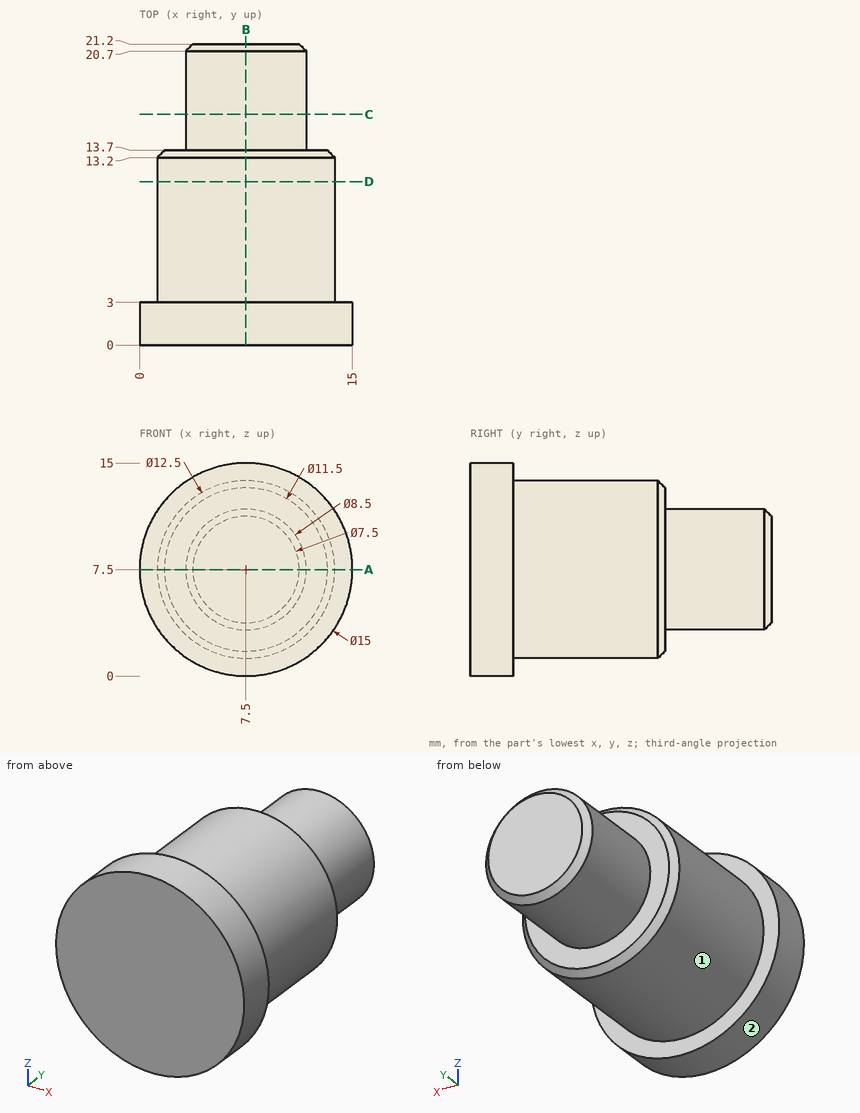
Design review of the part shown in the three views and the two pictorial views. Dimensions are in mm from the part's minimum x, y and z. A direction names the side the tool comes from. Give positions to 0.01 mm unless a question says otherwise; leave off trailing zeros. Write each loop counter-clockwise with the first axis right and the second up, starting at its lowest first coordinate (ties: lowest second). Pieces come first, ordered by that corner, then holes.
(1) Add section D-D (y = 11.5). Give the boundary of the cut face in (x, z).
Checked values:
outline: circle Ø12.5 at (7.5, 7.5)
(2) Add section A-A (z = 7.5). Give the boundary of the cut face in (x, y).
Checked values:
outline: (0, 0) - (15, 0) - (15, 3) - (13.75, 3) - (13.75, 13.2) - (13.25, 13.7) - (11.75, 13.7) - (11.75, 20.7) - (11.25, 21.2) - (3.75, 21.2) - (3.25, 20.7) - (3.25, 13.7) - (1.75, 13.7) - (1.25, 13.2) - (1.25, 3) - (0, 3) - close
(3) Clearance check with flat-ended pins moving along their axes: pin 1 Ø1.5 at (x, z) = (5, 3.5) entering from +Y; pin 2 Ø5 at (x, y) = (10, 16.5) entering from -Z; pin 3 Ø5 at (y, z) = (11.5, 7.5) entering from -X. State where each tip first meets the part, or that it passes through.
Checked values:
pin 1: stops at y = 20.98
pin 2: stops at z = 3.25
pin 3: stops at x = 1.25
(4) Tool access review of the marked faces 1 and 2: name each direction out of +Z, -Z, +X, -X, +Y, -Y from which nothing blocks a thin tool from reaching the whole face with its end or side.
Checked values:
face 1: +Y
face 2: +Y, -Y
(5) Add section C-C (y = 16.25). Give the boundary of the cut face in (x, z), and give its area (3 significant figures).
Checked values:
outline: circle Ø8.5 at (7.5, 7.5)
area: 56.7 mm2
(6) Add section B-B (x = 7.5). Give the boundary of the cut face in (y, z).
Checked values:
outline: (0, 0) - (3, 0) - (3, 1.25) - (13.2, 1.25) - (13.7, 1.75) - (13.7, 3.25) - (20.7, 3.25) - (21.2, 3.75) - (21.2, 11.25) - (20.7, 11.75) - (13.7, 11.75) - (13.7, 13.25) - (13.2, 13.75) - (3, 13.75) - (3, 15) - (0, 15) - close
(7) Wall thickness on line 1 along Y through (x, z) = (9.5, 12.5); line 2 along Y through (x, z) = (5, 14.25); line 3 along X through (y, z) = (5, 7.75) (3 decimals): over which ranges is each line inside the solid? List them lowest first.
Checked values:
line 1: y = 0 to 13.7
line 2: y = 0 to 3
line 3: x = 1.255 to 13.745
